For this review, take the finished solid that the model builds, in its own axes (mm). Face numbers are marked on the shaded views. Give positions to 0.01 mm unless a question says otherwise; leave off trailing zeros. Write each loop counter-clockwise with the first axis right and the second up, starting at its lowest first coordinate (ties: lowest second). Pieces come first, ordered by that corner, then holes. Notation, with made-up numbers: M 56,15.25 L 93,15.25 A11 cw 93,33.25 Z; hole C 49.5,-3 d1. An arc over 180 degrees is marked long. Use one line per item in the form item = value. Start each with the question number.
Q1. Consider section A-A on z = -46. Write out the cut boundary in (x, y).
Q2. Consider section C-C on x = -6. Write out the cut boundary in (y, z), and give its area (3 significant figures).
Q3. Consider section B-B on y = 0. Write out the cut boundary in (x, z), and give its area (3 significant figures).
Q4. Clearance check with flat-ended pins moving along their axes: pin 1 Ø9.5 at (x, z) = (22.63, -23.37) entering from +Y; pin 2 Ø18 at (x, y) = (-3, -8.5) entering from -Z; pin 3 Ø10 at (x, y) = (26.5, 44) entering from -Z. State where each tip first meets the part, or that it passes through.
Q5. Consider section D-D on x = 29. Write out the cut boundary in (y, z), and give its area (3 significant figures).
Q6. Mouldability with a two-part tool opening along Y and no side actions: class the marked faces 1, 2 and 3 as released by +Y, released by -Y, zero draft, split by the parting line, or undercut.
Q7. For probe 1 along Y at (x, z) = (0, 2); probe 2 along X at (y, z) = (-43.85, -46); probe 3 along Z at (x, y) = (-1.5, 50.5), list the stretches that pass through material, from the lowest coordinate up. Write a range as [from, to].
```python
from build123d import *
from build123d.topology import SkipClean

# Parameters (mm, degrees)
SKETCH1_W           = 70
SKETCH1_H           = 100
SKETCH1_R           = 8
BOSS_EXTRUDE1_DEPTH = 6
BOSS_EXTRUDE2_START = 10
SKETCH2_R           = 18
SKETCH2_R_2         = 8
BOSS_EXTRUDE2_DEPTH = 10
SKETCH3_W           = 70
SKETCH3_H           = 80
BOSS_EXTRUDE3_DEPTH = 6
SKETCH4_W           = 4.928950204
SKETCH4_H           = 5
CUT_EXTRUDE1_DEPTH  = 95.451045521
SKETCH5_R           = 3.006498603
SKETCH5_R_2         = 3
SKETCH5_R_3         = 25.009138209
CUT_EXTRUDE2_DEPTH  = 6


with BuildPart() as part:
    # Sketch1 → Boss-Extrude1 (new body)
    with BuildSketch(Plane.XY):
        with Locations((0, 10)):
            Rectangle(SKETCH1_W, SKETCH1_H)
        Circle(SKETCH1_R, mode=Mode.SUBTRACT)
    extrude(amount=BOSS_EXTRUDE1_DEPTH)

    # Sketch2 → Boss-Extrude2 (add)
    with SkipClean():  # the faces are left unmerged after this step: merging them gives an invalid solid
        with BuildSketch(Plane(origin=(0, 0, 0), x_dir=(-1, 0, 0), z_dir=(0, 0, -1)).offset(BOSS_EXTRUDE2_START)):
            with Locations(Location((0, 0, 0), (0, 0, 180))):
                Circle(SKETCH2_R)
            Circle(SKETCH2_R_2, mode=Mode.SUBTRACT)
        extrude(amount=-BOSS_EXTRUDE2_DEPTH)

    # Sketch3 → Boss-Extrude3 (add)
    with SkipClean():  # the faces are left unmerged after this step: merging them gives an invalid solid
        with BuildSketch(Plane.XZ.offset(40)):
            with Locations((0, -34)):
                Rectangle(SKETCH3_W, SKETCH3_H)
        extrude(amount=BOSS_EXTRUDE3_DEPTH)

    # Sketch4 → Cut-Extrude1 (cut, through all)
    with BuildSketch(Plane(origin=(0, 0, -10), x_dir=(-1, 0, 0), z_dir=(0, 0, -1))):
        with Locations((-7.535524898, 0)):
            Rectangle(SKETCH4_W, SKETCH4_H)
    extrude(amount=-CUT_EXTRUDE1_DEPTH, mode=Mode.SUBTRACT)

    # Sketch5 → Cut-Extrude2 (cut)
    with BuildSketch(Plane(origin=(0, -40, 0), x_dir=(1, 0, 0), z_dir=(0, 1, 0))):
        with Locations(Location((-22.627416998, 68.627416998, 0), (0, 0, 270))):
            Circle(SKETCH5_R)
        with Locations(Location((22.627416998, 68.627416998, 0), (0, 0, 270))):
            Circle(SKETCH5_R_2)
        with Locations(Location((22.627416998, 23.372583002, 0), (0, 0, 270))):
            Circle(SKETCH5_R_2)
        with Locations(Location((-22.627416998, 23.372583002, 0), (0, 0, 270))):
            Circle(SKETCH5_R_2)
        with Locations(Location((-0.009138209, 46.00000012, 0), (0, 0, 270))):
            Circle(SKETCH5_R_3)
    extrude(amount=-CUT_EXTRUDE2_DEPTH, mode=Mode.SUBTRACT)


solid = part.part
```
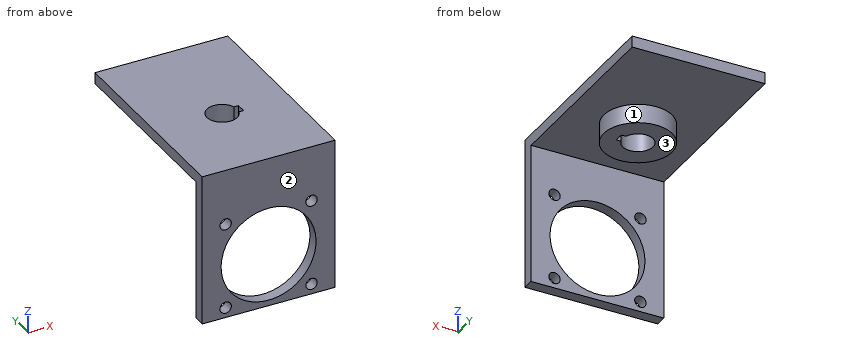
Working result:
q1.outline = M -35,-46 L -25.02,-46 L -25.02,-40 L -35,-40 Z; M 25,-46 L 35,-46 L 35,-40 L 25,-40 Z
q2.outline = M -46,-74 L -40,-74 L -40,-70.28 L -46,-70.28 Z; M -46,-21.72 L -40,-21.72 L -40,0 L -16.97,0 L -16.97,-10 L -5.29,-10 L -5.29,6 L -46,6 Z; M 5.29,-10 L 16.97,-10 L 16.97,0 L 60,0 L 60,6 L 5.29,6 Z
q2.area = 959 mm²
q3.outline = M -35,0 L -18,0 L -18,-10 L -8,-10 L -8,6 L -35,6 Z; M 10,-10 L 18,-10 L 18,0 L 35,0 L 35,6 L 10,6 Z
q3.area = 492 mm²
q4.pin_1 = -40
q4.pin_2 = -10
q4.pin_3 = 0
q5.outline = M -46,-74 L -40,-74 L -40,0 L 60,0 L 60,6 L -46,6 Z
q5.area = 1,080 mm²
q6.face_1 = undercut
q6.face_2 = released by -Y
q6.face_3 = zero draft
q7.probe_1 = [-46, -8], [8, 60]
q7.probe_2 = [-35, -25.02], [25, 35]
q7.probe_3 = [0, 6]
